Design review of the part built by this model. Coordinates are the model's own, in mm. A direction names the side the tool comes from. Coordinates: 2 decimals unless noted, no trailing zeros. Write each loop counter-clockwise with the first axis right and the second up, starting at its lowest first coordinate (ties: lowest second). Pieces come first, ordered by that corner, then holes.
Q1. Add section A-A, the plane z = 1.05. Give the number of separate pieces and of enclosed holes in the cut face, plus the area to 3 significant figures.
Q2. Add section B-B, the plane x = -235. Give the boundary of the cut face in (y, z).
Q3. The part is to be moulded in two halves that separate along Y. For faces 1 (the face through (210.367, 56.095, 2.958)), 2 (the face through (248.987, 58.813, 2.958)), 3 (the face through (-7, 61, 0)), say which applies: +Y half, -Y half, draft (parallel to the pull), parting line (faces both ways), or undercut.
Q4. Clearance check with flat-ended pins moving along their axes: pin 1 Ø12.5 at (x, y) = (-55, 25) entering from +Z; pin 2 Ø1.8 at (x, z) = (70.5, 4.5) entering from +Y; pin 3 Ø3 at (x, z) = (70.5, 2.5) entering from -Y; pin 4 Ø1.8 at (x, z) = (174.5, 4.5) entering from -Y. State where each tip first meets the part, or that it passes through.
Q5. Machinability: for faces 4 (the face through (-7, 61, 6)), 5 (the face through (-179.994, 59.45, 2.958)), which of the approach directions +Z, -Z, +X, -X, +Y, -Y give a long, thin tool a straight path to every point of the face, cutting with its end or side? Answer none if there is none.
Q6. Add section C-C, the plane y = 25. Give the boundary of the cut face in (x, z), plus the area to 3 significant figures.
Q7. To check wall thickness, follow probe 1 along Y at (x, z) = (-55, 2.3); probe 2 along Y at (x, z) = (-235, 2); probe 3 along X at (y, z) = (54.5, 2.1). State the ranges of each line that lie inside material, in increasing order.
Q8. Add section D-D, the plane x = 176. Give the boundary of the cut face in (y, z).
from build123d import *

# Parameters (mm, degrees)
SKETCH_1_R                   = 12.5
SKETCH_1_R_2                 = 7.5
EXTRUDE_1_DEPTH              = 6
HOLE_WIZARD_M6_1_D           = 7
HOLE_WIZARD_M6_1_CBORE_D     = 11
HOLE_WIZARD_M6_1_CBORE_DEPTH = 6.8
SKETCH_7_R                   = 4
CUT_EXTRUDE_1_DEPTH          = 10


with BuildPart() as part:
    # 草图1 → 凸台-拉伸1 (new body)
    with BuildSketch(Plane.XY):
        with BuildLine():
            Line((-255, 0), (45, 0))
            Line((45, 0), (115, 6))
            Line((115, 6), (195, 6))
            ThreePointArc((195, 6), (249, 60), (195, 114))
            Line((195, 114), (115, 114))
            Line((115, 114), (45, 120))
            Line((45, 120), (-235, 120))
            Line((-235, 120), (-255, 120))
            Line((-255, 120), (-255, 0))
        make_face()
        with Locations((-235, 100)):
            Circle(SKETCH_1_R, mode=Mode.SUBTRACT)
        with Locations((-235, 60)):
            Circle(SKETCH_1_R_2, mode=Mode.SUBTRACT)
        with BuildLine():
            Line((-155, 85), (-55, 85))
            ThreePointArc((-55, 85), (-30, 60), (-55, 35))
            Line((-55, 35), (-155, 35))
            ThreePointArc((-155, 35), (-180, 60), (-155, 85))
        make_face(mode=Mode.SUBTRACT)
        with BuildLine():
            Line((45, 85), (145, 85))
            ThreePointArc((145, 85), (170, 60), (145, 35))
            Line((145, 35), (45, 35))
            ThreePointArc((45, 35), (20, 60), (45, 85))
        make_face(mode=Mode.SUBTRACT)
    extrude(amount=EXTRUDE_1_DEPTH)

    # M6 六角圆柱头螺钉的柱形沉头孔1 (through all)
    with Locations(Plane.XY.offset(6)):
        with Locations((-55, 95), (-55, 25), (45, 95), (45, 25)):
            CounterBoreHole(HOLE_WIZARD_M6_1_D / 2, HOLE_WIZARD_M6_1_CBORE_D / 2, HOLE_WIZARD_M6_1_CBORE_DEPTH)

    # 草图7 → 切除-拉伸1 (cut)
    with BuildSketch(Plane(origin=(0, 0, 0), x_dir=(-1, 0, 0), z_dir=(0, 0, -1))):
        with Locations((-209.5, 60)):
            Circle(SKETCH_7_R)
    extrude(amount=-CUT_EXTRUDE_1_DEPTH, mode=Mode.SUBTRACT)


solid = part.part
Here are the results:
1. separate pieces: 1
1. enclosed holes: 9
1. area: 42,200 mm2
2. outline: (0, 0) - (52.5, 0) - (52.5, 6) - (0, 6) - close; (67.5, 0) - (87.5, 0) - (87.5, 6) - (67.5, 6) - close; (112.5, 0) - (120, 0) - (120, 6) - (112.5, 6) - close
3. face 1: undercut
3. face 2: parting line
3. face 3: draft
4. pin 1: stops at z = 6
4. pin 2: stops at y = 117.89
4. pin 3: stops at y = 2.06
4. pin 4: stops at y = 6
5. face 4: +Z, +X, -X, +Y, -Y
5. face 5: +Z, -Z
6. outline: (-255, 0) - (-60.5, 0) - (-60.5, 6) - (-255, 6) - close; (-49.5, 0) - (39.5, 0) - (39.5, 6) - (-49.5, 6) - close; (50.5, 0) - (236.12, 0) - (236.12, 6) - (50.5, 6) - close
6. area: 2,810 mm2
7. probe 1: y = 0 to 19.5, 30.5 to 35, 85 to 89.5, 100.5 to 120
7. probe 2: y = 0 to 52.5, 67.5 to 87.5, 112.5 to 120
7. probe 3: x = -255 to -240.1, -229.9 to -179.39, -30.61 to 20.61, 169.39 to 248.72
8. outline: (6, 0) - (114, 0) - (114, 6) - (6, 6) - close
